Check sheet for the modelled part. Datum: model origin and axes. Units: mm. Face numbers are marked on the shaded views. Coordinates: 2 decimals unless noted, no trailing zeros. Loops run counter-clockwise (first coordinate to the right, second up) from the corner with the lowest first, then second, coordinate; pieces in that order, holes last. Notation, with made-up numbers: (81.5, -33.5) -> (113.5, -33.5) arc R18 cw to (113.5, -16.5) -> close; hole circle Ø10 at (83, 25). An arc over 180 degrees is marked (long way). Use CSV: the item, a comma, the result in double quotes.
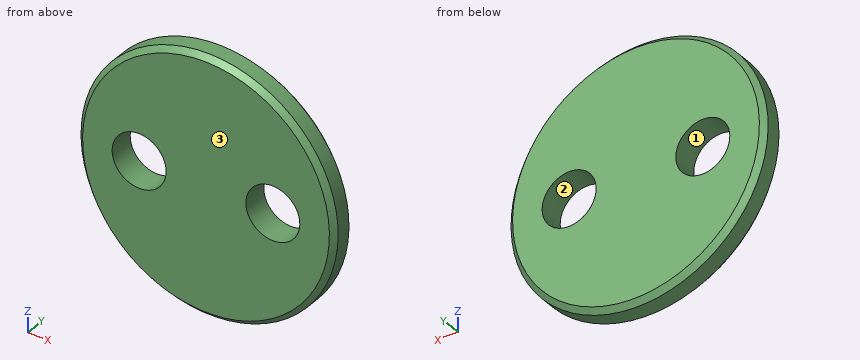
```python
from build123d import *

# Parameters (mm, degrees)
SKETCH1_R           = 25
SKETCH1_R_2         = 5.25
BOSS_EXTRUDE1_DEPTH = 5
CHAMFER1_SIZE       = 1


with BuildPart() as part:
    # Sketch1 → Boss-Extrude1 (new body)
    with BuildSketch(Plane(origin=(0, 0, 0), x_dir=(1, 0, 0), z_dir=(0, 1, 0))):
        with Locations(Location((0, 0, 0), (0, 0, 270))):
            Circle(SKETCH1_R)
        with Locations(Location((-13, 0, 0), (0, 0, 270))):
            Circle(SKETCH1_R_2, mode=Mode.SUBTRACT)
        with Locations(Location((13, 0, 0), (0, 0, 90))):
            Circle(SKETCH1_R_2, mode=Mode.SUBTRACT)
    extrude(amount=BOSS_EXTRUDE1_DEPTH)

    # Chamfer1
    chamfer1_edges = [part.edges().sort_by_distance(p)[0] for p in [
        (0, 0, -25),
        (0, 5, -25),
    ]]
    chamfer(chamfer1_edges, length=CHAMFER1_SIZE)


solid = part.part
```
1) Cross-section at B-B on y = 3.15. Record the boundary of the cut face in (x, z), and give its area (3 significant figures).
Answer below:
outline,"circle Ø50 at (0, 0); hole circle Ø10.5 at (-13, 0); hole circle Ø10.5 at (13, 0)"
area,"1,790 mm²"
2) Go/stop test with flat-tipped pins: pin 1 Ø1.5 at (x, y) = (-15, 3) entering from -Z; pin 2 Ø8.5 at (x, z) = (-13, 0) entering from +Y; pin 3 Ø2 at (x, y) = (1.5, 4) entering from -Z (3 decimals); pin 4 Ø1.5 at (y, z) = (4, 13) entering from +X. Record where each tip stops, or that it passes through.
Answer below:
pin 1,"stops at z = -20.54"
pin 2,"passes through"
pin 3,"stops at z = -24.995"
pin 4,"stops at x = 21.79"
3) Draft check along Z on the marked faces 1, 2 and 3. Enter one of: released by +Z, released by -Z, zero draft, split by the parting line, or undercut.
Answer below:
face 1,"undercut"
face 2,"undercut"
face 3,"zero draft"
4) Cross-section at A-A on z = 0. Record the boundary of the cut face in (x, y).
Answer below:
outline,"(-25, 1) -> (-24, 0) -> (-18.25, 0) -> (-18.25, 5) -> (-24, 5) -> (-25, 4) -> close; (-7.75, 0) -> (7.75, 0) -> (7.75, 5) -> (-7.75, 5) -> close; (18.25, 0) -> (24, 0) -> (25, 1) -> (25, 4) -> (24, 5) -> (18.25, 5) -> close"
5) Thickness scan on line 1 along X through (y, z) = (1.85, 0); line 2 along X through (y, z) = (0.5, 1.5); line 3 along Z through (x, y) = (-10.5, 4.8). Record the ranges inside material, lowest first. Write a range as from..to.
Answer below:
line 1,"x = -25..-18.25, -7.75..7.75, 18.25..25"
line 2,"x = -24.45..-18.03, -7.97..7.97, 18.03..24.45"
line 3,"z = -21.8..-4.62, 4.62..21.8"
